The drawing under review shows one solid part. Ordinate dimensions are in mm from its lowest x, y, z. A direction names the side the tool comes from. Give positions to 0.01 mm unless a question says otherwise; leave off trailing zeros. Order: outer loops, then holes, each group sorted by start corner. A loop starts at its lowest first (then second) coordinate and runs counter-clockwise, first axis right, second up. Notation, with made-up numbers: (86, 30.5) -> (109, 30.5) arc R15 cw to (109, 45.5) -> close; hole circle Ø1 at (12, -35.5). An arc over 180 degrees is marked (long way). One line per item, written item: value. Start each with the question number.
1) Consider section D-D (y = 16). State the section outline as (x, z) points.
2) Consider section B-B (z = 0.6). State the section outline as (x, y) points, plus the area to 3 significant figures.
3) For pin 1 (2 mm diameter, centred on x = 1.5, y = 20, fed in from -Z); pin 2 (2.5 mm diameter, centred on x = 4, y = 39, fed in from +Z); pin 3 (1.5 mm diameter, centred on y = 36, z = 1, fed in from -X); pin 4 (1 mm diameter, centred on x = 6, z = 2.5, fed in from +Y), all flat-tipped, find the tip position at first contact; note any pin that passes through.
4) Tool access review of the marked faces 4, 5, 6 and 7: name each direction out of +Z, -Z, +X, -X, +Y, -Y from which nothing blocks a thin tool from reaching the whole face with its end or side.
5) Consider section A-A (x = 4). State the section outline as (y, z) points.
6) The part is to be moulded in two halves that separate along X. For the marked faces 1, 2 and 3, say which applies: released by +X, released by -X, zero draft, split by the parting line, or undercut.
7) Consider section C-C (y = 5.5). State the section outline as (x, z) points, plus the area to 3 significant figures.
8) Wall thickness on line 1 along Y through (x, z) = (4, 1.15); line 2 along Y through (x, z) = (4.5, 2.85) (1 decimal); line 3 along X through (y, z) = (18, 1.8): over which ranges is each line inside the solid? List them lowest first. Write a range as from..to.
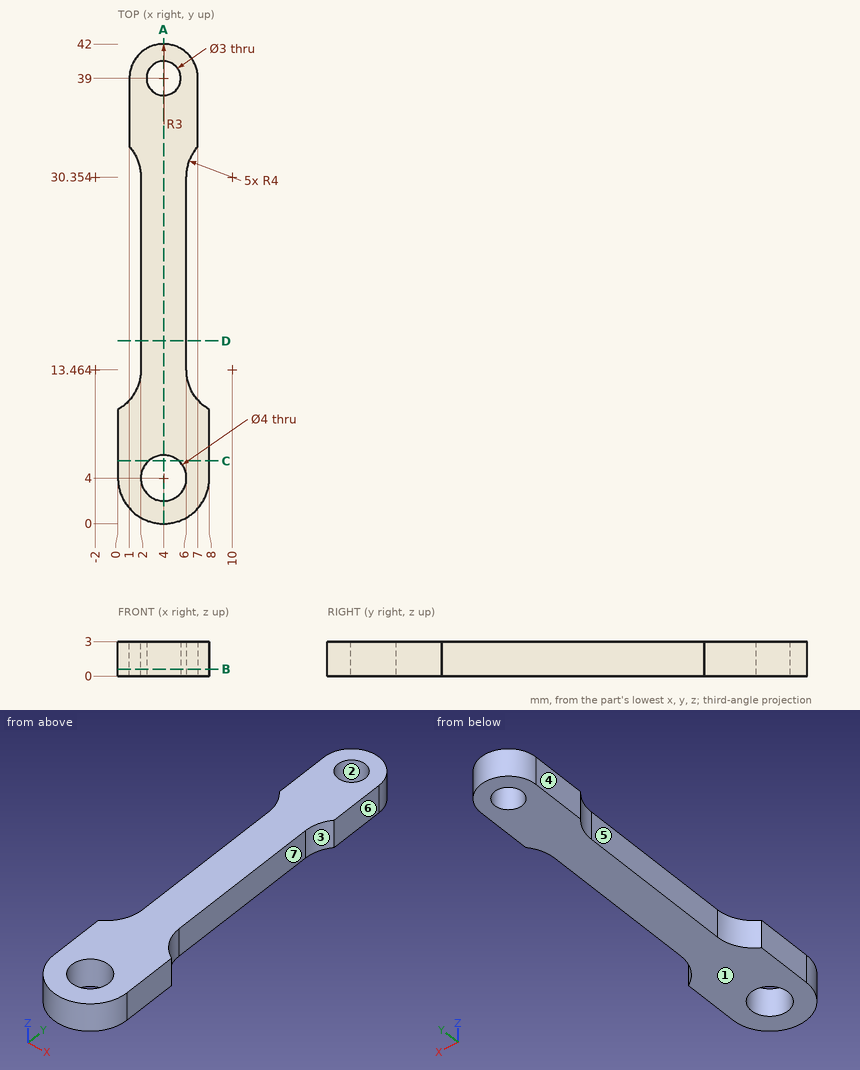
Checked values:
1. outline: (2, 0) -> (6, 0) -> (6, 3) -> (2, 3) -> close
2. outline: (0, 4) arc R4 ccw to (8, 4) -> (8, 10) arc R4 cw to (6, 13.46) -> (6, 30.35) arc R4 cw to (7, 33) -> (7, 39) arc R3 ccw to (1, 39) -> (1, 33) arc R4 cw to (2, 30.35) -> (2, 13.46) arc R4 cw to (0, 10) -> close; hole circle Ø4 at (4, 4); hole circle Ø3 at (4, 39)
2. area: 201 mm^2
3. pin 1: stops at z = 0
3. pin 2: passes through
3. pin 3: stops at x = 1
3. pin 4: stops at y = 41.6
4. face 4: +Z, -Z, -X, +Y
4. face 5: +Z, -Z, -X
4. face 6: +Z, -Z, +X, +Y
4. face 7: +Z, -Z, +X
5. outline: (0, 0) -> (2, 0) -> (2, 3) -> (0, 3) -> close; (6, 0) -> (37.5, 0) -> (37.5, 3) -> (6, 3) -> close; (40.5, 0) -> (42, 0) -> (42, 3) -> (40.5, 3) -> close
6. face 1: zero draft
6. face 2: undercut
6. face 3: released by +X
7. outline: (0, 0) -> (2.68, 0) -> (2.68, 3) -> (0, 3) -> close; (5.32, 0) -> (8, 0) -> (8, 3) -> (5.32, 3) -> close
7. area: 16.1 mm^2
8. line 1: y = 0..2, 6..37.5, 40.5..42
8. line 2: y = 0..2.1, 5.9..37.6, 40.4..42
8. line 3: x = 2..6
